Could you check a few things on this model? Use its own coordinates, in mm. A direction names the side the tool comes from. Give positions to 0.01 mm unless a question says otherwise; leave off trailing zeros. Loops run counter-clockwise (first coordinate to the right, second up) from the corner with the lowest first, then second, coordinate; pieces in that order, holes last.
1. For P1, Ø8, axis at x = 18, y = 51, coming from the -Z side; P2, Ø9.5, axis at x = -15, z = 295, coming from the +Y side; P3, Ø8, axis at x = 40.5, y = 190.5, coming from the -Z side; P4, Ø12, axis at x = -33.5, z = -189.5, coming from the +Y side, each with a flat end and sliding along its axis, tell me the tip position at first contact or that it passes through.
2. Imagine slicing it at A-A (z = -390). List the corners of the cut face in (x, y) for me.
3. Imagine slicing it at B-B (z = 491). List the corners of the cut face in (x, y) for me, plus the area to 3 significant figures.
4. Thinking about a two-plate mould opening in Z: for faces 4 (the cylindrical face through (-0.882, 28.735, 259.241)), 5 (the flat face through (1, 22, 431)), 6 (the conical face through (87.19, 233.14, 4.89)), which applies, +Z half, -Z half, draft (parallel to the pull), parting line (faces both ways), or undercut?
5. For faces 1 (the cylindrical face through (-1.26, 9.94, -242.74)), 2 (the flat face through (1, 22, -427)), 3 (the flat face through (-1, 1.2, 421)), which set-ups out of +Z, -Z, +X, -X, +Y, -Y let a thin tool reach every point of the face, with its end or its side?
6. I need wall thicknesses on line 1 along X through (y, z) = (6, -390); line 2 along Y through (x, z) = (18, 308.5); line 3 along Z through (x, y) = (27, 17.5). Which ranges of each line are inside material? Lowest first, please.
```python
from build123d import *

# Parameters (mm, degrees)
BOSS_EXTRUDE1_DEPTH     = 90
FILLET1_R               = 30
FILLET2_R               = 55
CUT_EXTRUDE1_DEPTH      = 640.147087923
CUT_EXTRUDE1_DEPTH_BACK = 640.147087923
SKETCH2_R               = 233
CUT_EXTRUDE2_DEPTH      = 640.147087923
CUT_EXTRUDE2_DEPTH_BACK = 640.147087923
SKETCH3_W               = 1220
SKETCH3_H               = 21.2
CUT_EXTRUDE3_DEPTH      = 27
MIRROR2_COPY_1_DEPTH    = 27
CUT_EXTRUDE4_DEPTH      = 640.147087923
CUT_EXTRUDE4_DEPTH_BACK = 640.147087923
SKETCH5_R               = 19
SKETCH5_R_2             = 6
CHAMFER1_SIZE           = 3


with BuildPart() as part:
    # Sketch1 → Boss-Extrude1 (new, symmetric)
    with BuildSketch(Plane(origin=(0, 0, 0), x_dir=(0, 0, -1), z_dir=(1, 0, 0))):
        with BuildLine():
            Line((-580, 22), (-252.041663223, 22))
            ThreePointArc((-252.041663223, 22), (0, 253), (252.041663223, 22))
            Line((252.041663223, 22), (580, 22))
            Line((580, 22), (580, -3))
            Line((580, -3), (227.980262304, -3))
            ThreePointArc((227.980262304, -3), (0, 228), (-227.980262304, -3))
            Line((-227.980262304, -3), (-580, -3))
            Line((-580, -3), (-580, 22))
        make_face()
    extrude(amount=BOSS_EXTRUDE1_DEPTH, both=True)

    # Fillet1
    fillet1_edges = [part.edges().sort_by_distance(p)[0] for p in [
        (0, 22, 252.041663223),
        (0, 22, -252.041663223),
    ]]
    fillet(fillet1_edges, radius=FILLET1_R)

    # Fillet2
    fillet2_edges = [part.edges().sort_by_distance(p)[0] for p in [
        (0, -3, -227.980262304),
        (0, -3, 227.980262304),
    ]]
    fillet(fillet2_edges, radius=FILLET2_R)

    # Sketch2 → Cut-Extrude1 (cut, two sides: drawn at the far end of the back side and taken through both)
    with BuildSketch(Plane(origin=(0, 0, 0), x_dir=(0, 0, -1), z_dir=(1, 0, 0)).offset(-CUT_EXTRUDE1_DEPTH_BACK)):
        Circle(SKETCH2_R)
    extrude(amount=CUT_EXTRUDE1_DEPTH + CUT_EXTRUDE1_DEPTH_BACK, mode=Mode.SUBTRACT)

    # Sketch3 → Cut-Extrude2 (cut, two sides: drawn at the far end of the back side and taken through both)
    with BuildSketch(Plane(origin=(0, 0, 0), x_dir=(0, 0, -1), z_dir=(1, 0, 0)).offset(-CUT_EXTRUDE2_DEPTH_BACK)):
        with Locations((0, -9.4)):
            Rectangle(SKETCH3_W, SKETCH3_H)
    extrude(amount=CUT_EXTRUDE2_DEPTH + CUT_EXTRUDE2_DEPTH_BACK, mode=Mode.SUBTRACT)

    # Sketch4 → Cut-Extrude3 (cut)
    with BuildSketch(Plane(origin=(90, 0, 0), x_dir=(0, 0, -1), z_dir=(1, 0, 0))):
        with BuildLine():
            Line((-598.01008044, 50), (-248.01008044, 50))
            ThreePointArc((-248.01008044, 50), (-252.546221213, 15.14615962), (-252.208247288, -20))
            Line((-252.208247288, -20), (-598.01008044, -20))
            Line((-598.01008044, -20), (-598.01008044, 50))
        make_face()
    cut_extrude3 = extrude(amount=-CUT_EXTRUDE3_DEPTH, mode=Mode.SUBTRACT)

    # Mirror1: Cut-Extrude3 across plane
    add(cut_extrude3.mirror(Plane.XY), mode=Mode.SUBTRACT)

    # Mirror2: Cut-Extrude3 across plane
    add(cut_extrude3.mirror(Plane(origin=(0, 0, 0), x_dir=(0, 0, 1), z_dir=(1, 0, 0))), mode=Mode.SUBTRACT)

    # Mirror2 copy 1 sketch → Mirror2 copy 1 (cut)
    with BuildSketch(Plane.ZY.offset(90)):
        with BuildLine():
            Line((-598.01008044, 50), (-248.01008044, 50))
            ThreePointArc((-248.01008044, 50), (-252.546221213, 15.14615962), (-252.208247288, -20))
            Line((-252.208247288, -20), (-598.01008044, -20))
            Line((-598.01008044, -20), (-598.01008044, 50))
        make_face()
    extrude(amount=-MIRROR2_COPY_1_DEPTH, mode=Mode.SUBTRACT)

    # Sketch5 → Cut-Extrude4 (cut, two sides: drawn at the far end of the back side and taken through both)
    with BuildSketch(Plane(origin=(0, 0, 0), x_dir=(1, 0, 0), z_dir=(0, 1, 0)).offset(-CUT_EXTRUDE4_DEPTH_BACK)):
        with Locations(Location((34, -390, 0), (0, 0, 90))):
            Circle(SKETCH5_R)
        with Locations(Location((34, 390, 0), (0, 0, 90))):
            Circle(SKETCH5_R)
        with Locations(Location((-34, -390, 0), (0, 0, 90))):
            Circle(SKETCH5_R)
        with Locations(Location((-34, 390, 0), (0, 0, 90))):
            Circle(SKETCH5_R)
        with Locations(Location((-15, -295, 0), (0, 0, 90))):
            Circle(SKETCH5_R_2)
        with Locations(Location((15, 295, 0), (0, 0, 90))):
            Circle(SKETCH5_R_2)
    extrude(amount=CUT_EXTRUDE4_DEPTH + CUT_EXTRUDE4_DEPTH_BACK, mode=Mode.SUBTRACT)

    # Chamfer1
    chamfer1_edges = [part.edges().sort_by_distance(p)[0] for p in [
        (-90, 233, 0),
        (90, 233, 0),
    ]]
    chamfer(chamfer1_edges, length=CHAMFER1_SIZE)


solid = part.part
```
Derived:
1. P1: stops at z = -248.6
1. P2: passes through
1. P3: stops at z = -170.96
1. P4: stops at y = 174.17
2. outline: (-63, 1.2) - (-53, 1.2) - (-53, 22) - (-63, 22) - close; (-15, 1.2) - (15, 1.2) - (15, 22) - (-15, 22) - close; (53, 1.2) - (63, 1.2) - (63, 22) - (53, 22) - close
3. outline: (-63, 1.2) - (63, 1.2) - (63, 22) - (-63, 22) - close
3. area: 2,620 mm2
4. face 4: +Z half
4. face 5: draft
4. face 6: undercut
5. face 1: +X, -X, -Y
5. face 2: -Z, +X, -X, +Y
5. face 3: +Z, -Z, +X, -X, -Y
6. line 1: x = -63 to -53, -15 to 15, 53 to 63
6. line 2: y = 1.2 to 22
6. line 3: z = -580 to -407.66, -372.34 to -235.35, 235.35 to 372.34, 407.66 to 580
